Read the model definition and answer for the solid it produces. Units are mm, in the model's axes. Face numbers are marked on the shaded views. A direction names the side the tool comes from. Round coordinates to 2 decimals unless told otherwise and drop trailing zeros. Order: outer loops, then holes, each group sorted by start corner. A loop starts at its lowest first (then second) coordinate and runs counter-clockwise, first axis right, second up.
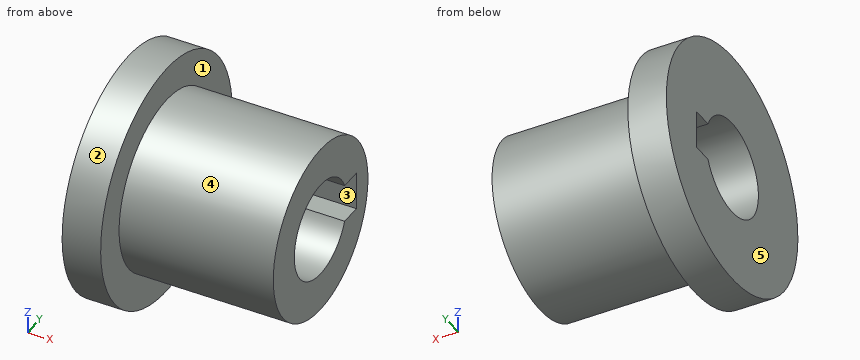
from build123d import *

# Parameters (mm, degrees)
SKETCH_2_W          = 4
SKETCH_2_H          = 6.8
CUT_EXTRUDE_1_DEPTH = 27.69269563


with BuildPart() as part:
    # 草图1 → 旋转1 (revolve)
    with BuildSketch(Plane.XY, mode=Mode.PRIVATE) as revolve_1_sk:
        Polygon((0, 5), (20, 5), (20, 9), (4, 9), (4, 12.5), (0, 12.5), align=None)
    revolve(revolve_1_sk.sketch.rotate(Axis((0, 0, 0), (1, 0, 0)), 90), axis=Axis((0, 0, 0), (1, 0, 0)))

    # 草图2 → 切除-拉伸1 (cut, through all)
    with BuildSketch(Plane.ZY):
        with Locations((0, 3.4)):
            Rectangle(SKETCH_2_W, SKETCH_2_H)
    extrude(amount=-CUT_EXTRUDE_1_DEPTH, mode=Mode.SUBTRACT)


solid = part.part
Q1. A cutting plane is placed at C-C, the plane x = 3.5. Give the vertices of the cut face in (y, z), plus the area to 3 significant figures.
Outcome:
outline: circle Ø25 at (0, 0); hole (4.58, -2) - (6.8, -2) - (6.8, 2) - (4.58, 2) arc R5 ccw (long way) to start
area: 405 mm2
Q2. Flat-ended cylindrical pins translate along their axes: pin 1 (2.5 mm diameter, centred on x = 9, y = 6, fed in from +Z); pin 2 (6 mm diameter, centred on x = 14, z = 1, fed in from +Y); pin 3 (8 mm diameter, centred on x = 12.5, y = 10, fed in from +Z). Find the tip coordinate at first contact, or state that the pin passes through.
Outcome:
pin 1: stops at z = 7.64
pin 2: stops at y = 9
pin 3: stops at z = 6.71
Q3. Straight lines are drawn through the part: probe 1 along Y at (x, z) = (9.5, 0); probe 2 along Y at (x, z) = (1.25, -0.25); probe 3 along X at (y, z) = (10.75, 5.75). For each, find the intervals that lie inside material, in ascending order.
Outcome:
probe 1: y = -9 to -5, 6.8 to 9
probe 2: y = -12.5 to -4.99, 6.8 to 12.5
probe 3: x = 0 to 4
Q4. For a pull along Y with two mould halves and no side action, classify the marked faces 1, 2 and 3 as released by +Y, released by -Y, zero draft, split by the parting line, or undercut.
Outcome:
face 1: zero draft
face 2: split by the parting line
face 3: undercut
Q5. For the marked faces 4 and 5, determine the directions among +Z, -Z, +X, -X, +Y, -Y from which every point of the face is accessible in a straight line to the end or side of a thin tool.
Outcome:
face 4: +X
face 5: +Z, -Z, -X, +Y, -Y
Q6. A cutting plane is placed at B-B, the plane z = 0. Give the vertices of the cut face in (x, y).
Outcome:
outline: (0, -12.5) - (4, -12.5) - (4, -9) - (20, -9) - (20, -5) - (0, -5) - close; (0, 6.8) - (20, 6.8) - (20, 9) - (4, 9) - (4, 12.5) - (0, 12.5) - close
Q7. A cutting plane is placed at D-D, the plane z = -7. Give the vertices of the cut face in (x, y), plus the area to 3 significant figures.
Outcome:
outline: (0, -10.36) - (4, -10.36) - (4, -5.66) - (20, -5.66) - (20, 5.66) - (4, 5.66) - (4, 10.36) - (0, 10.36) - close
area: 264 mm2
Q8. A cutting plane is placed at A-A, the plane y = 0. Give the vertices of the cut face in (x, z), plus the area to 3 significant figures.
Outcome:
outline: (0, -12.5) - (4, -12.5) - (4, -9) - (20, -9) - (20, -5) - (0, -5) - close; (0, 5) - (20, 5) - (20, 9) - (4, 9) - (4, 12.5) - (0, 12.5) - close
area: 188 mm2
